Verification items for the finished model (mm, model axes). A direction names the side the tool comes from. Round coordinates to 2 decimals unless told otherwise and drop trailing zeros. Loops run counter-clockwise (first coordinate to the right, second up) from the corner with the lowest first, then second, coordinate; pieces in that order, holes last.
from build123d import *

# Parameters (mm, degrees)
SKETCH_1_R          = 2
EXTRUDE_1_DEPTH     = 10
SKETCH_2_R          = 3.5
EXTRUDE_2_DEPTH     = 4
CUT_EXTRUDE_1_DEPTH = 2
CHAMFER_1_SIZE      = 0.5
SKETCH_4_R          = 0.75
CUT_EXTRUDE_2_DEPTH = 13.980754986


with BuildPart() as part:
    # 草图1 → 凸台-拉伸1 (new body)
    with BuildSketch(Plane.XY):
        Circle(SKETCH_1_R)
    extrude(amount=EXTRUDE_1_DEPTH)

    # 草图2 → 凸台-拉伸2 (add)
    with BuildSketch(Plane.XY.offset(10)):
        Circle(SKETCH_2_R)
    extrude(amount=EXTRUDE_2_DEPTH)

    # 草图3 → 切除-拉伸1 (cut)
    with BuildSketch(Plane.XY.offset(14)):
        Polygon((-0.863155152, 1.501653483), (-1.73204764, 0.003312453), (-0.868892488, -1.498341031), (0.863155152, -1.501653483), (1.73204764, -0.003312453), (0.868892488, 1.498341031), align=None)
    extrude(amount=-CUT_EXTRUDE_1_DEPTH, mode=Mode.SUBTRACT)

    # 倒角1
    chamfer_1_edges = [part.edges().sort_by_distance(p)[0] for p in [
        (-2, 0, 0),
    ]]
    chamfer(chamfer_1_edges, length=CHAMFER_1_SIZE)

    # 草图4 → 切除-拉伸2 (cut, through all)
    with BuildSketch(Plane.XY.offset(12)):
        Circle(SKETCH_4_R)
    extrude(amount=-CUT_EXTRUDE_2_DEPTH, mode=Mode.SUBTRACT)


solid = part.part
1. Release check for a two-part mould opening along Y. For faces 1 (the face through (0, -2, 5)), 2 (the face through (2, -2, 10)), 3 (the face through (-1.307, -0.737, 13.014)) record: released by +Y, released by -Y, zero draft, split by the parting line, or undercut.
2. Scan lines: L1, parallel to Y at x = 0, z = 8.5; L2, parallel to Z at x = 0.5, y = 1.25; L3, parallel to Z at x = -2.25, y = 1.5. Record each from-to range of solid material in increasing order.
3. Section check B-B (z = 10.25). Enter the section's corners in (x, y), then the cut area to 3 significant figures.
4. Section check A-A (x = 0). Enter the section's corners in (y, z).
5. Section check C-C (y = -2.75). Enter the section's corners in (x, z), then the cut area to 3 significant figures.
6. Gauge pin test, flat ends, axial feed: P1, Ø2.5, axis at x = 0, y = 0, coming from the +Z side; P2, Ø1, axis at y = 2, z = 11.5, coming from the +X side; P3, Ø1.5, axis at x = 2, z = 7.5, coming from the -Y side. Record the tip position at first contact, or that the pin passes through.
7. Tool access check on faces 4 (the face through (-1, 0, 0)), 5 (the face through (-1.292, 0.763, 13.014)). Record the directions out of +Z, -Z, +X, -X, +Y, -Y that give a thin tool (end or side, any length) a straight path to the whole face; none if there is none.
8. Section check D-D (z = 3). Enter the section's corners in (x, y).
Taken from the geometry:
1. face 1: split by the parting line
1. face 2: zero draft
1. face 3: undercut
2. L1: y = -2 to -0.75, 0.75 to 2
2. L2: z = 0 to 12
2. L3: z = 10 to 14
3. outline: circle Ø7 at (0, 0); hole circle Ø1.5 at (0, 0)
3. area: 36.7 mm2
4. outline: (-3.5, 10) - (-2, 10) - (-2, 0.5) - (-1.5, 0) - (-0.75, 0) - (-0.75, 12) - (-1.5, 12) - (-1.5, 14) - (-3.5, 14) - close; (0.75, 0) - (1.5, 0) - (2, 0.5) - (2, 10) - (3.5, 10) - (3.5, 14) - (1.5, 14) - (1.5, 12) - (0.75, 12) - close
5. outline: (-2.17, 10) - (2.17, 10) - (2.17, 14) - (-2.17, 14) - close
5. area: 17.3 mm2
6. P1: stops at z = 12
6. P2: stops at x = 3.16
6. P3: stops at y = -1.56
7. face 4: -Z, +X, -X, +Y, -Y
7. face 5: +Z
8. outline: circle Ø4 at (0, 0); hole circle Ø1.5 at (0, 0)
